Input: part model. Units: mm. Frame: model coordinates. Face numbers are marked on the shaded views. A direction names the side the tool comes from. Coordinates: 2 decimals unless noted, no trailing zeros. Loops run counter-clockwise (first coordinate to the right, second up) from the corner with the lowest first, then second, coordinate; pieces in that order, holes last. Notation, with made-up numbers: (-26.5, 70.25) -> (13.5, 70.25) arc R19 cw to (13.5, 78.25) -> close; hole circle Ø11 at (80.25, 80). An arc over 180 degrees is marked (long way). Answer as a JSON object with one key per item and string values.
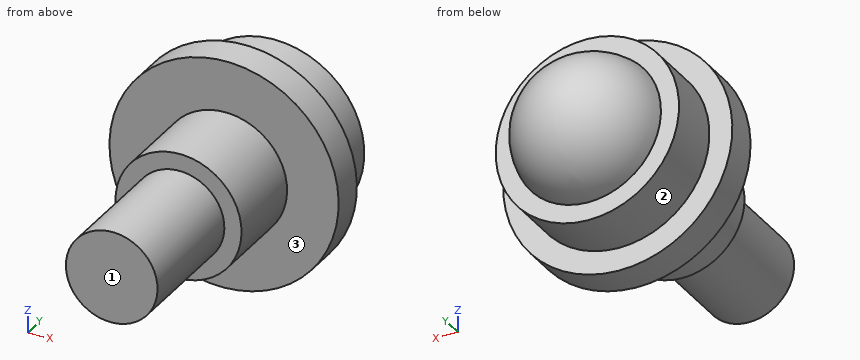
from build123d import *

# Parameters (mm, degrees)
SKETCH2_R           = 11
BOSS_EXTRUDE1_DEPTH = 15
SKETCH3_R           = 8
BOSS_EXTRUDE2_DEPTH = 22


with BuildPart() as part:
    # Sketch1 → Revolve1 (revolve)
    with BuildSketch(Plane.XY, mode=Mode.PRIVATE) as revolve1_sk:
        with BuildLine():
            Line((-12.845232579, 16), (-16, 16))
            Line((-16, 16), (-16, 6))
            Line((-16, 6), (-20, 6))
            Line((-20, 6), (-20, 0))
            Line((-20, 0), (0, 0))
            Line((0, 0), (0, 27))
            ThreePointArc((0, 27), (-8.455767263, 23.874208829), (-12.845232579, 16))
        make_face()
    revolve(revolve1_sk.sketch.rotate(Axis((0, 0, 0), (0, 1, 0)), 270), axis=Axis((0, 0, 0), (0, 1, 0)))

    # Sketch2 → Boss-Extrude1 (add)
    with BuildSketch(Plane(origin=(0, 0, 0), x_dir=(-1, 0, 0), z_dir=(0, -1, 0))):
        with Locations(Location((0, 0, 0), (0, 0, 90))):
            Circle(SKETCH2_R)
    extrude(amount=BOSS_EXTRUDE1_DEPTH)

    # Sketch3 → Boss-Extrude2 (add)
    with BuildSketch(Plane(origin=(0, -15, 0), x_dir=(-1, 0, 0), z_dir=(0, -1, 0))):
        with Locations(Location((0, 0, 0), (0, 0, 90))):
            Circle(SKETCH3_R)
    extrude(amount=BOSS_EXTRUDE2_DEPTH)


solid = part.part
1. Section query C-C (y = 13). Return loops of the section in (x, z).
Reply:
{"outline": "circle Ø32 at (0, 0)"}
2. Section query D-D (x = 14). Return loops of the section in (y, z).
Reply:
{"outline": "(0, -14.28) -> (6, -14.28) -> (6, -7.75) -> (16, -7.75) -> (16, 7.75) -> (6, 7.75) -> (6, 14.28) -> (0, 14.28) -> close"}
3. Pin query (flat end, axial travel): P1, Ø16, axis at x = -7.5, z = 1.5, coming from the +Y side; P2, Ø4, axis at y = -30, z = 2.5, coming from the -X side; P3, Ø2, axis at y = 0, z = -11.5, coming from the -X side; P4, Ø10, axis at y = -15.5, z = 14.5, coming from the -X side. Return the tip coordinate at first contact, or that it passes through.
Reply:
{"P1": "stops at y = 27", "P2": "stops at x = -7.98", "P3": "stops at x = -17.02", "P4": "stops at x = -5.5"}
4. Section query A-A (x = 0). Return loops of the section in (y, z), plus the area to 3 significant figures.
Reply:
{"outline": "(-37, -8) -> (-15, -8) -> (-15, -11) -> (0, -11) -> (0, -20) -> (6, -20) -> (6, -16) -> (16, -16) -> (16, -12.85) arc R13 ccw to (16, 12.85) -> (16, 16) -> (6, 16) -> (6, 20) -> (0, 20) -> (0, 11) -> (-15, 11) -> (-15, 8) -> (-37, 8) -> close", "area": "1,460 mm2"}
5. Access query for the marked faces 1, 2 and 3. Directions: +Z, -Z, +X, -X, +Y, -Y. A direction counts if a zero-diameter tool reaches every point of the face in a straight line with its end or side. Return the directions, or none.
Reply:
{"face 1": "+Z, -Z, +X, -X, -Y", "face 2": "+Y", "face 3": "-Y"}
6. Section query B-B (z = 0). Return loops of the section in (x, y).
Reply:
{"outline": "(-20, 0) -> (-11, 0) -> (-11, -15) -> (-8, -15) -> (-8, -37) -> (8, -37) -> (8, -15) -> (11, -15) -> (11, 0) -> (20, 0) -> (20, 6) -> (16, 6) -> (16, 16) -> (12.85, 16) arc R13 ccw to (-12.85, 16) -> (-16, 16) -> (-16, 6) -> (-20, 6) -> close"}
7. Line query: line 1 along Z through (x, y) = (0.5, 13.5); line 2 along Y through (x, z) = (17, 4.5); line 3 along Y through (x, z) = (-13, 5). Output: solid intervals per line, ascending.
Reply:
{"line 1": "z = -15.99 to 15.99", "line 2": "y = 0 to 6", "line 3": "y = 0 to 16"}
